For this review, take the finished solid that the model builds, in its own axes (mm). A direction names the side the tool comes from. Coordinates: 2 decimals unless noted, no trailing zeros. Loops run counter-clockwise (first coordinate to the right, second up) from the corner with the lowest first, then second, coordinate; pieces in that order, holes last.
1. Take a section at A-A, the plane x = 10.5. State the section outline as (y, z) points.
2. Mouldability with a two-part tool opening along X and no side actions: class faces 3 (the face through (8.6, 0.5, -3.5)), 4 (the face through (20.48, 0.49, 0.08)), 5 (the face through (4.44, 0.49, 0.03)) as pulls with the +X half, pulls with the -X half, needs draft (parallel to the pull), parting line crosses it, or undercut.
3. Take a section at C-C, the plane y = 0.65. State the section outline as (x, z) points.
4. Take a section at D-D, the plane z = -3. State the section outline as (x, y) points, then the cut area to 3 significant figures.
5. Clearance check with a flat-ended pin moving along its axis: P1, Ø1.9, axis at x = 16.98, z = 0, coming from the +Y side (3 decimals). State where the tip first meets the part, or that it passes through.
6. Take a section at B-B, the plane z = 0. State the section outline as (x, y) points, then the cut area to 3 significant figures.
7. Machinability: for faces 1 (the face through (-3.5, 0.5, -0.1)), 2 (the face through (8.5, 0.5, -1.55)), which of the approach directions +Z, -Z, +X, -X, +Y, -Y give a long, thin tool a straight path to every point of the face, cutting with its end or side? Answer none if there is none.
8. To check wall thickness, follow probe 1 along X at (y, z) = (0.2, 0); probe 2 along Z at (x, y) = (8.25, 0.6); probe 3 along X at (y, z) = (0.25, 0.25). State the ranges of each line that lie inside material, in increasing order.
```python
from build123d import *

# Parameters (mm, degrees)
SKETCH_1_R      = 1.55
EXTRUDE_1_DEPTH = 1


with BuildPart() as part:
    # 草图1 → 凸台-拉伸1 (new body)
    with BuildSketch(Plane(origin=(0, 0, 0), x_dir=(1, 0, 0), z_dir=(0, 1, 0))):
        with BuildLine():
            ThreePointArc((0, 3.5), (-3.5, 0), (0, -3.5))
            Line((0, -3.5), (16.98, -3.5))
            ThreePointArc((16.98, -3.5), (20.48, 0), (16.98, 3.5))
            Line((16.98, 3.5), (0, 3.5))
        make_face()
        with Locations(Location((0, 0, 0), (0, 0, 270))):
            Circle(SKETCH_1_R, mode=Mode.SUBTRACT)
        with BuildLine():
            ThreePointArc((10.99, 1.55), (12.54, 0), (10.99, -1.55))
            Line((10.99, -1.55), (5.99, -1.55))
            ThreePointArc((5.99, -1.55), (4.44, 0), (5.99, 1.55))
            Line((5.99, 1.55), (10.99, 1.55))
        make_face(mode=Mode.SUBTRACT)
        with Locations(Location((16.98, 0, 0), (0, 0, 270))):
            Circle(SKETCH_1_R, mode=Mode.SUBTRACT)
    extrude(amount=EXTRUDE_1_DEPTH)


solid = part.part
```
Results list:
1. outline: (0, -3.5) - (1, -3.5) - (1, -1.55) - (0, -1.55) - close; (0, 1.55) - (1, 1.55) - (1, 3.5) - (0, 3.5) - close
2. face 3: needs draft
2. face 4: pulls with the +X half
2. face 5: undercut
3. outline: (0, -3.5) - (16.98, -3.5) arc R3.5 ccw to (16.98, 3.5) - (0, 3.5) arc R3.5 ccw to start; hole circle Ø3.1 at (0, 0); hole (5.99, -1.55) - (10.99, -1.55) arc R1.55 ccw to (10.99, 1.55) - (5.99, 1.55) arc R1.55 ccw to start; hole circle Ø3.1 at (16.98, 0)
4. outline: (-1.8, 0) - (18.78, 0) - (18.78, 1) - (-1.8, 1) - close
4. area: 20.6 mm2
5. P1: passes through
6. outline: (-3.5, 0) - (-1.55, 0) - (-1.55, 1) - (-3.5, 1) - close; (1.55, 0) - (4.44, 0) - (4.44, 1) - (1.55, 1) - close; (12.54, 0) - (15.43, 0) - (15.43, 1) - (12.54, 1) - close; (18.53, 0) - (20.48, 0) - (20.48, 1) - (18.53, 1) - close
6. area: 9.68 mm2
7. face 1: -X, +Y, -Y
7. face 2: +Y, -Y
8. probe 1: x = -3.5 to -1.55, 1.55 to 4.44, 12.54 to 15.43, 18.53 to 20.48
8. probe 2: z = -3.5 to -1.55, 1.55 to 3.5
8. probe 3: x = -3.49 to -1.53, 1.53 to 4.46, 12.52 to 15.45, 18.51 to 20.47
